Verification items for the finished model (mm, model axes). A direction names the side the tool comes from. Round coordinates to 2 decimals unless told otherwise and drop trailing zeros. Write each loop counter-clockwise with the first axis right and the second up, starting at its lowest first coordinate (ties: lowest second). Pieces come first, ordered by that corner, then holes. Notation, with made-up numbers: (-21, 8) -> (30, 8) arc R29 ccw to (30, 46) -> close; hole circle Ø11 at (10.25, -4). An arc over 180 degrees is marked (long way). Answer as a JSON object with one key per item and string values. Group by question number.
(1) Scan lines: L1, parallel to Y at x = 3.5, z = -25; L2, parallel to Y at x = 1, z = 26; L3, parallel to Z at x = 19, y = 23.5. Record each from-to range of solid material in increasing order. Write a range as from..to.
(2) Sectioned sample at B-B on y = 0. Record the cut outline in (x, z), and give its area (3 significant figures).
(3) Sectioned sample at A-A on z = 0. Record the cut outline in (x, y), and give its area (3 significant figures).
(4) Sectioned sample at D-D on z = 25. Record the cut outline in (x, y), and give its area (3 significant figures).
(5) Set-up check for faces 1 (the face through (5.423, 0.198, -29.496)), 2 (the face through (15.563, 0.33, 7.493)): record each of +Z, -Z, +X, -X, +Y, -Y from which the full face is reachable in a straight line by a thin tool's end or side.
(6) Sectioned sample at C-C on x = 4.25. Record the cut outline in (y, z), and give its area (3 significant figures).
(7) Gauge pin test, flat ends, axial feed: pin 1 Ø10.5 at (y, z) = (0, -25) entering from +X; pin 2 Ø2 at (y, z) = (16.5, -15.5) entering from -X. Record the tip position at first contact, or that the pin passes through.
(8) Draft check along Y on faces 3 (the face through (10, 0, -50)), 4 (the face through (11, 0, -30)), 5 (the face through (10, 40, 1)). Enter one of: released by +Y, released by -Y, zero draft, split by the parting line, or undercut.
```python
from build123d import *

# Parameters (mm, degrees)
SKETCH_1_W                = 100
SKETCH_1_H                = 80
EXTRUDE_1_DEPTH           = 20
HOLE_WIZARD_M8_1_D        = 6.8
HOLE_WIZARD_1_D           = 9
HOLE_WIZARD_1_CBORE_D     = 15
HOLE_WIZARD_1_CBORE_DEPTH = 9
CHAMFER_1_SIZE            = 5


with BuildPart() as part:
    # 草图1 → 凸台-拉伸1 (new body)
    with BuildSketch(Plane(origin=(0, 0, 0), x_dir=(0, 0, -1), z_dir=(1, 0, 0))):
        Rectangle(SKETCH_1_W, SKETCH_1_H)
    extrude(amount=EXTRUDE_1_DEPTH)

    # M8 螺纹孔1 (through all)
    with Locations(Plane(origin=(20, 0, 0), x_dir=(0, 0, -1), z_dir=(1, 0, 0))):
        with Locations((-24.748737342, 24.748737342), (24.748737342, 24.748737342), (24.748737342, -24.748737342), (-24.748737342, -24.748737342)):
            Hole(HOLE_WIZARD_M8_1_D / 2)

    # 打孔尺寸(%根据)内六角圆柱头螺钉的类型1 (through all)
    with Locations(Plane(origin=(20, 0, 0), x_dir=(0, 0, -1), z_dir=(1, 0, 0))):
        with Locations((-25, 0), (0, 0), (25, 0)):
            CounterBoreHole(HOLE_WIZARD_1_D / 2, HOLE_WIZARD_1_CBORE_D / 2, HOLE_WIZARD_1_CBORE_DEPTH)

    # 倒角1
    chamfer_1_edges = [part.edges().sort_by_distance(p)[0] for p in [
        (10, -40, -50),
        (10, -40, 50),
        (10, 40, 50),
        (10, 40, -50),
    ]]
    chamfer(chamfer_1_edges, length=CHAMFER_1_SIZE)


solid = part.part
```
Computed values:
{
 "1": {"L1": "-40..-28.14, -21.36..-4.5, 4.5..21.36, 28.14..40", "L2": "-40..-27.91, -21.59..-4.39, 4.39..21.59, 27.91..40", "L3": "-50..-27.91, -21.59..21.59, 27.91..50"},
 "2": {"outline": "(0, -50) -> (20, -50) -> (20, -32.5) -> (11, -32.5) -> (11, -29.5) -> (0, -29.5) -> close; (0, -20.5) -> (11, -20.5) -> (11, -17.5) -> (20, -17.5) -> (20, -7.5) -> (11, -7.5) -> (11, -4.5) -> (0, -4.5) -> close; (0, 4.5) -> (11, 4.5) -> (11, 7.5) -> (20, 7.5) -> (20, 17.5) -> (11, 17.5) -> (11, 20.5) -> (0, 20.5) -> close; (0, 29.5) -> (11, 29.5) -> (11, 32.5) -> (20, 32.5) -> (20, 50) -> (0, 50) -> close", "area": "1,300 mm2"},
 "3": {"outline": "(0, -40) -> (20, -40) -> (20, -7.5) -> (11, -7.5) -> (11, -4.5) -> (0, -4.5) -> close; (0, 4.5) -> (11, 4.5) -> (11, 7.5) -> (20, 7.5) -> (20, 40) -> (0, 40) -> close", "area": "1,370 mm2"},
 "4": {"outline": "(0, -40) -> (20, -40) -> (20, -28.14) -> (0, -28.14) -> close; (0, -21.36) -> (20, -21.36) -> (20, -7.5) -> (11, -7.5) -> (11, -4.5) -> (0, -4.5) -> close; (0, 4.5) -> (11, 4.5) -> (11, 7.5) -> (20, 7.5) -> (20, 21.36) -> (0, 21.36) -> close; (0, 28.14) -> (20, 28.14) -> (20, 40) -> (0, 40) -> close", "area": "1,090 mm2"},
 "5": {"face 1": "+X, -X", "face 2": "+X"},
 "6": {"outline": "(-40, -45) -> (-35, -50) -> (35, -50) -> (40, -45) -> (40, 45) -> (35, 50) -> (-35, 50) -> (-40, 45) -> close; hole circle Ø6.8 at (-24.75, -24.75); hole circle Ø6.8 at (-24.75, 24.75); hole circle Ø9 at (0, -25); hole circle Ø9 at (0, 0); hole circle Ø9 at (0, 25); hole circle Ø6.8 at (24.75, -24.75); hole circle Ø6.8 at (24.75, 24.75)", "area": "7,610 mm2"},
 "7": {"pin 1": "x = 11", "pin 2": "x = 0"},
 "8": {"face 3": "zero draft", "face 4": "undercut", "face 5": "released by +Y"}
}
